from build123d import *

# Parameters (mm, degrees)
BLOCK_BODY_DEPTH            = 40
CROSS_HOLE_SKETCH_R         = 4.5
CROSS_HOLE_DEPTH            = 87.622762369
RECTANGULAR_CUT_SKETCH_W    = 25
RECTANGULAR_CUT_SKETCH_H    = 25
RECTANGULAR_CUT_15X75_DEPTH = 87.622762369
TOP_CLAMP_HOLE_SKETCH_R     = 5.5
TOP_CLAMP_HOLE_DEPTH        = 18.5


with BuildPart() as part:
    # Block Profile Sketch → Block Body (new body)
    with BuildSketch(Plane.XY):
        with BuildLine():
            Line((-58.339548854, 25), (-58.339548854, 0))
            Line((-58.339548854, 0), (41.660451146, 0))
            Line((41.660451146, 0), (41.660451146, 20))
            Line((41.660451146, 20), (23.660451146, 20))
            Line((23.660451146, 20), (23.660451146, 28.5))
            Line((23.660451146, 28.5), (-3.52361978, 28.5))
            ThreePointArc((-3.52361978, 28.5), (-27.42950068, 30), (-3.52361978, 31.5))
            Line((-3.52361978, 31.5), (23.660451146, 31.5))
            Line((23.660451146, 31.5), (23.660451146, 50))
            Line((23.660451146, 50), (-15.038278665, 50))
            Line((-15.038278665, 50), (-58.339548854, 25))
        make_face()
    extrude(amount=BLOCK_BODY_DEPTH)

    # Cross Hole Sketch → Cross Hole (cut, through all)
    with BuildSketch(Plane.XY.offset(40)):
        with Locations((-45.339548854, 12)):
            Circle(CROSS_HOLE_SKETCH_R)
    extrude(amount=-CROSS_HOLE_DEPTH, mode=Mode.SUBTRACT)

    # Rectangular Cut Sketch → Rectangular Cut 15x75 (cut, through all)
    with BuildSketch(Plane.XZ):
        with Locations((-45.839548854, 27.5)):
            Rectangle(RECTANGULAR_CUT_SKETCH_W, RECTANGULAR_CUT_SKETCH_H)
    extrude(amount=-RECTANGULAR_CUT_15X75_DEPTH, mode=Mode.SUBTRACT)

    # Top Clamp Hole Sketch → Top Clamp Hole (cut)
    with BuildSketch(Plane(origin=(0, 50, 0), x_dir=(1, 0, 0), z_dir=(0, 1, 0))):
        with Locations(Location((16.660451146, -20, 0), (0, 0, 270))):
            Circle(TOP_CLAMP_HOLE_SKETCH_R)
    extrude(amount=-TOP_CLAMP_HOLE_DEPTH, mode=Mode.SUBTRACT)


solid = part.part
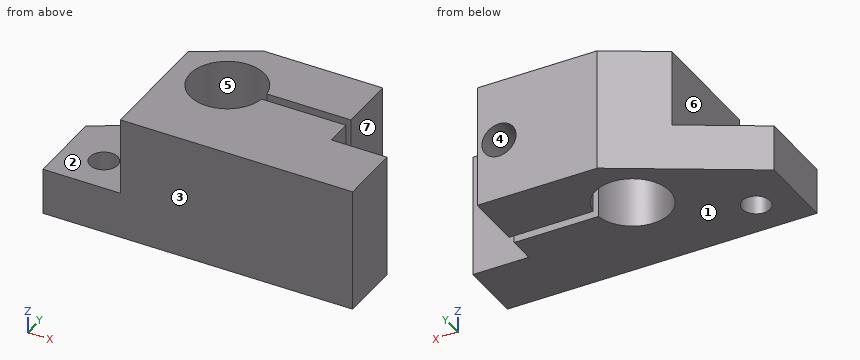
Geometry: final body of the model. Coordinates: model frame, mm. Face numbers are marked on the shaded views. A direction names the side the tool comes from. Coordinates: 2 decimals unless noted, no trailing zeros. Order: outer loops, then holes, each group sorted by start corner. A loop starts at its lowest first (then second) coordinate and runs counter-clockwise, first axis right, second up.
(1) Section query C-C (x = -8). Return the cut outline in (y, z).
(2) Section query B-B (y = 12). Return the cut outline in (x, z), plus the area to 3 significant figures.
(3) Section query A-A (z = 20). Return the cut outline in (x, y).
(4) First-contact query: pin 1 (20.5 mm diameter, centred on y = 43, z = 13, fed in from +X); pin 2 (7 mm diameter, centred on x = -45.34, y = 12, fed in from +Z); pin 3 (6 mm diameter, centred on x = 19.5, y = 9.5, fed in from -Z); pin 4 (9 mm diameter, centred on x = 33.5, z = 28.5, fed in from +Y). Flat tips, straight axial feed; report the tip coordinate or a pass-through.
(5) Access query for the marked faces 5, 6 and 7. Directions: +Z, -Z, +X, -X, +Y, -Y. A direction counts if a zero-diameter tool reaches every point of the face in a straight line with its end or side. Return the directions, or none.
(6) Draft query along Z for the marked faces 1, 2, 3 and 4. Return one class per face: pulls with the +Z half, pulls with the -Z half, needs draft (parallel to the pull), parting line crosses it, or undercut.
(7) Material intervals for probe 1 along X at (y, z) = (33, 16); probe 2 along Y at (x, z) = (12, 28.5); probe 3 along Y at (x, z) = (25.5, 34), sorted ascending.
(8) Section query D-D (y = 38). Return the cut outline in (x, z).
Solution:
1. outline: (0, 0) - (20.58, 0) - (20.58, 40) - (0, 40) - close; (39.42, 0) - (50, 0) - (50, 40) - (39.42, 40) - close
2. outline: (-58.34, 0) - (-49.84, 0) - (-49.84, 15) - (-58.34, 15) - close; (-40.84, 0) - (41.66, 0) - (41.66, 40) - (-33.34, 40) - (-33.34, 15) - (-40.84, 15) - close
2. area: 3,240 mm2
3. outline: (-33.34, 0) - (41.66, 0) - (41.66, 20) - (23.66, 20) - (23.66, 28.5) - (-3.52, 28.5) arc R12 cw (long way) to (-3.52, 31.5) - (11.16, 31.5) - (11.16, 50) - (-15.04, 50) - (-33.34, 39.43) - close; (22.16, 31.5) - (23.66, 31.5) - (23.66, 50) - (22.16, 50) - close
4. pin 1: stops at x = 23.66
4. pin 2: passes through
4. pin 3: stops at z = 0
4. pin 4: stops at y = 20
5. face 5: +Z, -Z
5. face 6: +Z, -X, +Y, -Y
5. face 7: +Z, -Z, +X, +Y
6. face 1: pulls with the -Z half
6. face 2: pulls with the +Z half
6. face 3: needs draft
6. face 4: undercut
7. probe 1: x = -33.34 to -27.05, -3.81 to 12.89, 20.44 to 23.66
7. probe 2: y = 0 to 28.5, 31.5 to 50
7. probe 3: y = 0 to 20
8. outline: (-35.82, 0) - (-24.37, 0) - (-24.37, 40) - (-33.34, 40) - (-33.34, 15) - (-35.82, 15) - close; (-6.49, 0) - (23.66, 0) - (23.66, 40) - (-6.49, 40) - close; hole circle Ø11 at (16.66, 20)
